```python
from build123d import *

# Parameters (mm, degrees)
EXTRUDE_1_DEPTH     = 4
SKETCH_4_R          = 10.89
SKETCH_4_R_2        = 5
CUT_EXTRUDE_1_DEPTH = 0.5
CUT_EXTRUDE_1_DRAFT = -60
CHAMFER_2_SIZE      = 0.333333333


with BuildPart() as part:
    # 草图3 → 凸台-拉伸1 (new body)
    with BuildSketch(Plane(origin=(0, 0, 0), x_dir=(0, 0, -1), z_dir=(1, 0, 0))):
        Polygon((5, 2.886751346), (0, 5.773502692), (-5, 2.886751346), (-5, -2.886751346), (0, -5.773502692), (5, -2.886751346), align=None)
    extrude(amount=EXTRUDE_1_DEPTH)


with BuildPart() as cut_extrude_1_tool:
    # 草图4 → 切除-拉伸1 (with draft: the straight prism first)
    with BuildSketch(Plane.ZY):
        Circle(SKETCH_4_R)
        Circle(SKETCH_4_R_2, mode=Mode.SUBTRACT)
    extrude(amount=-CUT_EXTRUDE_1_DEPTH)
    # 切除-拉伸1: the draft: its side faces are tilted about the plane it starts from
    cut_extrude_1_sides = [cut_extrude_1_tool.faces().sort_by_distance(p)[0] for p in [
        (0.25, 0, -10.89),
        (0.25, 0, -5),
    ]]
    draft(cut_extrude_1_sides, Plane.ZY, CUT_EXTRUDE_1_DRAFT)


with BuildPart() as part_1:
    add(part.part)

    # 切除-拉伸1: cut by cut_extrude_1_tool
    add(cut_extrude_1_tool.part, mode=Mode.SUBTRACT)

    # 草图5 → 旋转1 (revolve)
    with BuildSketch(Plane.XY, mode=Mode.PRIVATE) as revolve_1_sk:
        with BuildLine():
            Line((4.6, 3), (16, 3))
            Line((16, 3), (16, 0))
            Line((16, 0), (4, 0))
            Line((4, 0), (4, 3.6))
            ThreePointArc((4, 3.6), (4.175735931, 3.175735931), (4.6, 3))
        make_face()
    revolve(revolve_1_sk.sketch.rotate(Axis((4, 0, 0), (1, 0, 0)), 180), axis=Axis((4, 0, 0), (1, 0, 0)))

    # 倒角2
    chamfer_2_edges = [part_1.edges().sort_by_distance(p)[0] for p in [
        (16, 3, 0),
    ]]
    chamfer(chamfer_2_edges, length=CHAMFER_2_SIZE)


solid = part_1.part
```
Here's how the part is built. I have some questions about the finished solid (model axes, mm). A direction names the side the tool comes from. Round coordinates to 2 decimals unless told otherwise and drop trailing zeros. Order: outer loops, then holes, each group sorted by start corner. A loop starts at its lowest first (then second) coordinate and runs counter-clockwise, first axis right, second up. Notation, with made-up numbers: M 17,60.25 L 33,60.25 A17 cw 33,66.25 Z; hole C 35,46 d9. An arc over 180 degrees is marked long. One line per question, with ' | ' between items.
1) For faces 1 (the face through (10.21, -2.86, -0.9)), 2 (the face through (0.106, 5.184, 0.013)), which set-ups out of +Z, -Z, +X, -X, +Y, -Y let a thin tool reach every point of the face, with its end or its side?
Working result:
face 1: +X | face 2: -X, +Y
2) For pin 1 Ø3 at (y, z) = (-3, -3) entering from +X; pin 2 Ø5 at (x, z) = (7, 1.5) entering from +Y, each with a flat end and sliding along its axis, tell me the tip position at first contact or that it passes through.
Working result:
pin 1: x = 15.92 | pin 2: y = 3
3) I need wall thicknesses on line 1 along X through (y, z) = (4.5, 0); line 2 along Z through (x, y) = (3.75, 5); line 3 along Y through (x, z) = (4.75, 0.5). Which ranges of each line are inside material? Lowest first, please.
Working result:
line 1: 0 to 4 | line 2: -1.34 to 1.34 | line 3: -2.96 to 2.96
4) I want a section at A-A, the plane x = 10.5. Write out the boundary of the cut face in (y, z), then the cut area to 3 significant figures.
Working result:
outline: C 0,0 d6 | area: 28.3 mm²
